from build123d import *

# Parameters (mm, degrees)
BOSS_EXTRUDE1_DEPTH = 8
FILLET1_R           = 10


with BuildPart() as part:
    # Sketch1 → Boss-Extrude1 (new body)
    with BuildSketch(Plane.XY):
        Polygon((0, 0), (80, 0), (141.28355545, -51.423008775), (154.139307643, -36.102119913), (87.279404685, 20), (0, 20), align=None)
    extrude(amount=BOSS_EXTRUDE1_DEPTH)

    # Fillet1
    fillet1_edges = [part.edges().sort_by_distance(p)[0] for p in [
        (0, 20, 4),
        (87.279404685, 20, 4),
        (154.139307643, -36.102119913, 4),
    ]]
    fillet(fillet1_edges, radius=FILLET1_R)


solid = part.part
Geometry check sheet. Reference: the model listing, model coordinates, mm. A direction names the side the tool comes from. Round coordinates to 2 decimals unless told otherwise and drop trailing zeros. Loops run counter-clockwise (first coordinate to the right, second up) from the corner with the lowest first, then second, coordinate; pieces in that order, holes last. Notation, with made-up numbers: (66, -20.75) -> (73, -20.75) arc R29 ccw to (73, 1.25) -> close; hole circle Ø6 at (89.5, 61.5). An arc over 180 degrees is marked (long way). Answer as a JSON object with one key per item and string values. Group by question number.
Item 1: Set-up check for faces 1 (the face through (87.11, 19.38, 4.06)), 2 (the face through (39, 0, 4)): record each of +Z, -Z, +X, -X, +Y, -Y from which the full face is reachable in a straight line by a thin tool's end or side.
Item 2: Thickness scan on line 1 along Y through (x, z) = (17.5, 5); line 2 along X through (y, z) = (-29, 0.75); line 3 along X through (y, z) = (-19, 1.25). Record the ranges inside material, lowest first.
Item 3: Cross-section at C-C, the plane y = -14. Record the cut outline in (x, z), plus the area to 3 significant figures.
Item 4: Depth check by flat-ended pin: pin 1 Ø4 at (x, z) = (33, 4.5) entering from -Y; pin 2 Ø1.5 at (y, z) = (-28.5, 4) entering from +X; pin 3 Ø1.5 at (y, z) = (0.5, 3.5) entering from +X. Enter the tip coordinate at first touch or a pass-through.
Item 5: Cross-section at A-A, the plane z = 3.75. Record the cut outline in (x, y), plus the area to 3 significant figures.
Item 6: Cross-section at B-B, the plane x = 129.5. Record the cut outline in (y, z), plus the area to 3 significant figures.
Determined:
{
 "1": {"face 1": "+Z, -Z, +X, +Y", "face 2": "+Z, -Z, -X, -Y"},
 "2": {"line 1": "y = 0 to 20", "line 2": "x = 114.56 to 145.68", "line 3": "x = 102.64 to 133.76"},
 "3": {"outline": "(96.68, 0) -> (127.8, 0) -> (127.8, 8) -> (96.68, 8) -> close", "area": "249 mm²"},
 "4": {"pin 1": "stops at y = 0", "pin 2": "stops at x = 145.97", "pin 3": "stops at x = 111.41"},
 "5": {"outline": "(0, 0) -> (80, 0) -> (141.28, -51.42) -> (147.71, -43.76) arc R10 ccw to (146.48, -29.67) -> (90.07, 17.66) arc R10 ccw to (83.64, 20) -> (10, 20) arc R10 ccw to (0, 10) -> close", "area": "3,300 mm²"},
 "6": {"outline": "(-41.54, 0) -> (-15.43, 0) -> (-15.43, 8) -> (-41.54, 8) -> close", "area": "209 mm²"}
}
